Part model, mm, in its own coordinate system. Face numbers are marked on the shaded views. Coordinates: 2 decimals unless noted, no trailing zeros. Write each loop counter-clockwise with the first axis right and the second up, starting at its lowest first coordinate (ties: lowest second). Pieces come first, ordered by that corner, then holes. Notation, with made-up numbers: M 14,-32 L 63,-32 A21 cw 63,-15 Z; hole C -29.75,65 d3. An arc over 180 degrees is marked long. Use a Markdown table: item, result. Add a question column.
Q1. Slice it at C-C on z = 6. Write the cut outline in (x, y), then the cut area to 3 significant figures.
Q2. Wall check: L1, parallel to Y at x = 75, z = 4.75; L2, parallel to X at y = -183, z = 13; L3, parallel to Y at x = 86.5, z = 12.75. Give the ranges that are in metal, low to high. Write a range as from..to.
Q3. Slice it at A-A on y = -95. Write the cut outline in (x, z), then the cut area to 3 significant figures.
Q4. Slice it at D-D on y = -140. Write the cut outline in (x, z), then the cut area to 3 significant figures.
Q5. Mould opens along Y. For the marked faces 1, 2, 3 and 4 say: released by +Y, released by -Y, zero draft, split by the parting line, or undercut.
Q6. Slice it at B-B on x = 75. Write the cut outline in (y, z), then the cut area to 3 significant figures.
Q7. Pin check, flat tips, straight feed: pin 1 Ø1.5 at (y, z) = (-122, 17.5) entering from -X; pin 2 Ø6 at (y, z) = (-105.5, 14) entering from +X. Stop position of each tip, or through.
from build123d import *

# Parameters (mm, degrees)
SKETCH1_R              = 20
BOSS_EXTRUDE1_DEPTH    = 20
M12_TAPPED_HOLE1_D     = 10.2
M12_TAPPED_HOLE1_DEPTH = 29.25
M12_TAPPED_HOLE1_TIP   = 3.064389157
CHAMFER1_SIZE          = 1.5


with BuildPart() as part:
    # Sketch1 → Boss-Extrude1 (new body)
    with BuildSketch(Plane.XY):
        Polygon((0, 0), (150, 0), (150, -60), (110, -200), (40, -200), (0, -60), align=None)
        with Locations((75, -140)):
            Circle(SKETCH1_R, mode=Mode.SUBTRACT)
    extrude(amount=BOSS_EXTRUDE1_DEPTH)

    # M12 Tapped Hole1
    with Locations(Plane.XY.offset(20)):
        with Locations((75, -95), (75, -185)):
            Hole(M12_TAPPED_HOLE1_D / 2, depth=M12_TAPPED_HOLE1_DEPTH)
            with Locations((0, 0, -(M12_TAPPED_HOLE1_DEPTH + M12_TAPPED_HOLE1_TIP / 2))):  # 118° drill point
                Cone(0, M12_TAPPED_HOLE1_D / 2, M12_TAPPED_HOLE1_TIP, mode=Mode.SUBTRACT)

    # Chamfer1
    chamfer1_edges = [part.edges().sort_by_distance(p)[0] for p in [
        (55, -140, 0),
        (55, -140, 20),
    ]]
    chamfer(chamfer1_edges, length=CHAMFER1_SIZE)


solid = part.part
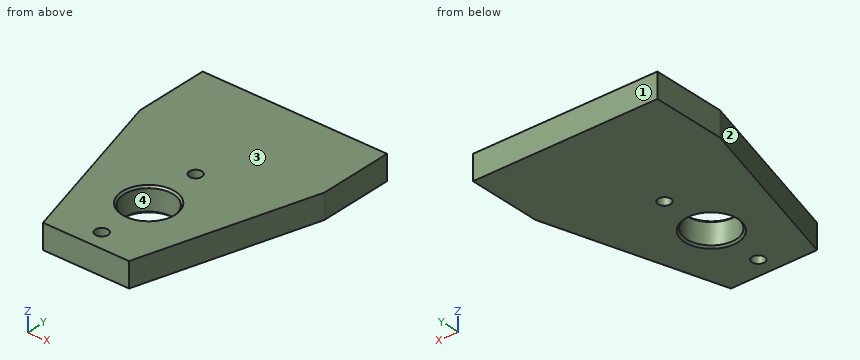
Recorded:
| question | item | result |
|---|---|---|
| 1 | outline | M 0,-60 L 40,-200 L 110,-200 L 150,-60 L 150,0 L 0,0 Z; hole C 75,-140 d40; hole C 75,-185 d10.2; hole C 75,-95 d10.2 |
| 1 | area | 23,000 mm² |
| 2 | L1 | -200..-190.1, -179.9..-160, -120..-100.1, -89.9..0 |
| 2 | L2 | 35.14..70.31, 79.69..114.86 |
| 2 | L3 | -200..-156.36, -123.64..0 |
| 3 | outline | M 10,0 L 69.9,0 L 69.9,20 L 10,20 Z; M 80.1,0 L 140,0 L 140,20 L 80.1,20 Z |
| 3 | area | 2,400 mm² |
| 4 | outline | M 22.86,0 L 53.5,0 L 55,1.5 L 55,18.5 L 53.5,20 L 22.86,20 Z; M 95,1.5 L 96.5,0 L 127.14,0 L 127.14,20 L 96.5,20 L 95,18.5 Z |
| 4 | area | 1,280 mm² |
| 5 | face 1 | released by +Y |
| 5 | face 2 | released by -Y |
| 5 | face 3 | zero draft |
| 5 | face 4 | undercut |
| 6 | outline | M -200,0 L -190.1,0 L -190.1,20 L -200,20 Z; M -179.9,0 L -161.5,0 L -160,1.5 L -160,18.5 L -161.5,20 L -179.9,20 Z; M -120,1.5 L -118.5,0 L -100.1,0 L -100.1,20 L -118.5,20 L -120,18.5 Z; M -89.9,0 L 0,0 L 0,20 L -89.9,20 Z |
| 6 | area | 2,790 mm² |
| 7 | pin 1 | x = 17.5 |
| 7 | pin 2 | x = 137.86 |
